Verification items for the finished model (mm, model axes). A direction names the side the tool comes from. Give positions to 0.01 mm unless a question says otherwise; leave off trailing zeros. Order: outer loops, then holes, each group sorted by start corner. A loop starts at its lowest first (then second) coordinate and runs counter-clockwise, first axis right, second up. Notation, with made-up numbers: (54.25, 28) - (98.25, 28) arc R35 ccw to (98.25, 60) - close; hole circle Ø1 at (-5.75, 83). An arc over 180 degrees is marked (long way). Answer as a JSON object with one key per item and string values.
```python
from build123d import *

# Parameters (mm, degrees)
GB_T_6728_2002_SQUARE_HOLLOW_SECTION_60_DEPTH = 1272
CUT_EXTRUDE1_DEPTH                            = 1274.767639721
CUT_EXTRUDE1_DEPTH_BACK                       = 1274.767639721


with BuildPart() as part:
    # Sketch1 → GB/T 6728-2002 square hollow section 60×60×4(1) (new body)
    with BuildSketch(Plane(origin=(0, 0, 0), x_dir=(-1, 0, 0), z_dir=(0, 1, 0))):
        with BuildLine():
            Line((-22, -30), (22, -30))
            ThreePointArc((22, -30), (27.656854249, -27.656854249), (30, -22))
            Line((30, -22), (30, 22))
            ThreePointArc((30, 22), (27.656854249, 27.656854249), (22, 30))
            Line((22, 30), (-22, 30))
            ThreePointArc((-22, 30), (-27.656854249, 27.656854249), (-30, 22))
            Line((-30, 22), (-30, -22))
            ThreePointArc((-30, -22), (-27.656854249, -27.656854249), (-22, -30))
        make_face()
        with BuildLine():
            Line((-22, -26), (22, -26))
            ThreePointArc((22, -26), (24.828427125, -24.828427125), (26, -22))
            Line((26, -22), (26, 22))
            ThreePointArc((26, 22), (24.828427125, 24.828427125), (22, 26))
            Line((22, 26), (-22, 26))
            ThreePointArc((-22, 26), (-24.828427125, 24.828427125), (-26, 22))
            Line((-26, 22), (-26, -22))
            ThreePointArc((-26, -22), (-24.828427125, -24.828427125), (-22, -26))
        make_face(mode=Mode.SUBTRACT)
    extrude(amount=GB_T_6728_2002_SQUARE_HOLLOW_SECTION_60_DEPTH)

    # Sketch2 → Cut-Extrude1 (cut, two sides: drawn at the far end of the back side and taken through both)
    with BuildSketch(Plane.XY.offset(30).offset(-CUT_EXTRUDE1_DEPTH_BACK)):
        Polygon((-30, 1272), (30, 1204.468946968), (30, 1272), align=None)
        Polygon((-30, 0), (-30, 67.531053032), (30, 0), align=None)
    extrude(amount=CUT_EXTRUDE1_DEPTH + CUT_EXTRUDE1_DEPTH_BACK, mode=Mode.SUBTRACT)


solid = part.part
```
(1) Section check A-A (z = -8.5). Record the cut outline in (x, y).
Computed values:
{"outline": "(-30, 67.53) - (-26, 63.03) - (-26, 1267.5) - (-30, 1272) - close; (26, 4.5) - (30, 0) - (30, 1204.47) - (26, 1208.97) - close"}
(2) Access from +Z, -Z, +X, -X, +Y, -Y to the whole of each face (thin tool, end or side, straight path). Record for faces 4 (the flat face through (26, 598, 0)), 5 (the flat face through (30, 594, 0)).
Computed values:
{"face 4": "+Y, -Y", "face 5": "+Z, -Z, +X, +Y, -Y"}
(3) Release check for a two-part mould opening along X. For faces 1 (the flat face through (-0.42, 34.24, -27.09)), 2 (the flat face through (0, 627, -26)), 3 (the flat face through (-0.42, 1238.71, -27.09)) record: pulls with the +X half, pulls with the -X half, needs draft (parallel to the pull), parting line crosses it, or undercut.
Computed values:
{"face 1": "pulls with the -X half", "face 2": "undercut", "face 3": "pulls with the +X half"}
(4) Section check C-C (x = 1). Record the cut outline in (y, z).
Computed values:
{"outline": "(32.64, -30) - (1237.11, -30) - (1237.11, -26) - (32.64, -26) - close; (32.64, 26) - (1237.11, 26) - (1237.11, 30) - (32.64, 30) - close"}
(5) Section check B-B (y = 210.5). Record the cut outline in (x, z), then the cut area to 3 significant figures.
Computed values:
{"outline": "(-30, -22) arc R8 ccw to (-22, -30) - (22, -30) arc R8 ccw to (30, -22) - (30, 22) arc R8 ccw to (22, 30) - (-22, 30) arc R8 ccw to (-30, 22) - close; hole (-26, -22) arc R4 ccw to (-22, -26) - (22, -26) arc R4 ccw to (26, -22) - (26, 22) arc R4 ccw to (22, 26) - (-22, 26) arc R4 ccw to (-26, 22) - close", "area": "855 mm²"}
(6) Gauge pin test, flat end, axial feed: pin 1 Ø3 at (x, z) = (-23, 14.5) entering from +Y. Record the tip position at first contact, or that the pin passes through.
Computed values:
{"pin 1": "passes through"}
(7) Material ranges on line 1 along X through (y, z) = (932, 3.5); line 2 along Z through (x, y) = (-24, 416.5), recorded low to high. Write a range as [from, to].
Computed values:
{"line 1": "x = [-30, -26], [26, 30]", "line 2": "z = [-29.75, -25.46], [25.46, 29.75]"}
